from build123d import *

# Parameters (mm, degrees)
CUT_EXTRUDE1_START      = 8
CUT_EXTRUDE1_DEPTH      = 1.5
CUT_EXTRUDE2_DEPTH      = 140.867794721
CUT_EXTRUDE2_DEPTH_BACK = 140.867794721
SKETCH3_R               = 4


with BuildPart() as part:
    # Sketch1 → Revolve2 (revolve)
    with BuildSketch(Plane.XY, mode=Mode.PRIVATE) as revolve2_sk:
        Polygon((0, 8), (44, 8), (44, 10), (114, 10), (114, 11), (139, 11), (139, 4), (94, 4), (94, 0), (0, 0), align=None)
    revolve(revolve2_sk.sketch.rotate(Axis((0, 0, 0), (1, 0, 0)), 90), axis=Axis((0, 0, 0), (1, 0, 0)))

    # Sketch2 → Cut-Extrude1 (cut)
    with BuildSketch(Plane(origin=(0, 0, 0), x_dir=(1, 0, 0), z_dir=(0, 1, 0)).offset(CUT_EXTRUDE1_START)):
        with BuildLine():
            Line((23, 2), (41, 2))
            ThreePointArc((41, 2), (43, 0), (41, -2))
            Line((41, -2), (23, -2))
            ThreePointArc((23, -2), (21, 0), (23, 2))
        make_face()
    extrude(amount=-CUT_EXTRUDE1_DEPTH, mode=Mode.SUBTRACT)

    # Sketch3 → Cut-Extrude2 (cut, two sides: drawn at the far end of the back side and taken through both)
    with BuildSketch(Plane(origin=(0, 0, 0), x_dir=(1, 0, 0), z_dir=(0, 1, 0)).offset(-CUT_EXTRUDE2_DEPTH_BACK)):
        with Locations(Location((94, 0, 0), (0, 0, 270))):
            Circle(SKETCH3_R)
    extrude(amount=CUT_EXTRUDE2_DEPTH + CUT_EXTRUDE2_DEPTH_BACK, mode=Mode.SUBTRACT)


solid = part.part
The model under review builds one solid part; all positions refer to its coordinate system, in mm. A direction names the side the tool comes from. Give positions to 0.01 mm unless a question says otherwise; leave off trailing zeros. Order: outer loops, then holes, each group sorted by start corner. A loop starts at its lowest first (then second) coordinate and runs counter-clockwise, first axis right, second up. Notation, with made-up numbers: M 87.5,77.5 L 94.5,77.5 A16 cw 94.5,102.5 Z; hole C -17.75,19.5 d2. An arc over 180 degrees is marked long. Answer in a Markdown table with one row per item. Add a question column.
1. Add section B-B on y = 0. State the section outline as (x, z) points, plus the area to 3 significant figures.
2. For pin 1 Ø3 at (x, z) = (88, -4.5) entering from +Y; pin 2 Ø7 at (y, z) = (0, 0) entering from +X; pin 3 Ø9 at (x, z) = (94, 0) entering from -Y, all flat-tipped, find the tip position at first contact; note any pin that passes through.
3. Machinability: for faces 1 (the flat face through (0, 0, 0)), 2 (the flat face through (114, 10, -2)), 3 (the cylindrical face through (116.185, 1.532, 3.695)), which of the approach directions +Z, -Z, +X, -X, +Y, -Y give a long, thin tool a straight path to every point of the face, cutting with its end or side? Answer none if there is none.
4. Add section A-A on z = 0. State the section outline as (x, y) points, plus the area to 3 significant figures.
5. Mouldability with a two-part tool opening along X and no side actions: class faces 4 (the flat face through (44, -8.2, 0)), 5 (the flat face through (139, 5, 0)), 6 (the cylindrical face through (79.49, -3, 9.54)), 7 (the flat face through (32, 6.5, 0)) as released by +X, released by -X, zero draft, split by the parting line, or undercut.
6. To check wall thickness, follow line 1 along X through (y, z) = (-5.5, 0); line 2 along Z through (x, y) = (94, 0.5); line 3 along Y through (x, z) = (122.5, 0). State the ranges of each line that lie inside material, in increasing order.
7. Add section C-C on y = -6.25. State the section outline as (x, z) points.
8. Add section D-D on x = 83.5. State the section outline as (y, z) points.
The answers:
| question | item | result |
|---|---|---|
| 1 | outline | M 0,-8 L 44,-8 L 44,-10 L 114,-10 L 114,-11 L 139,-11 L 139,-4 L 94,-4 A4 cw 94,4 L 139,4 L 139,11 L 114,11 L 114,10 L 44,10 L 44,8 L 0,8 Z |
| 1 | area | 2,270 mm2 |
| 2 | pin 1 | y = 9.54 |
| 2 | pin 2 | x = 92.06 |
| 2 | pin 3 | y = -10 |
| 3 | face 1 | +Z, -Z, -X, +Y, -Y |
| 3 | face 2 | -X |
| 3 | face 3 | +X |
| 4 | outline | M 0,-8 L 44,-8 L 44,-10 L 90,-10 L 90,10 L 44,10 L 44,8 L 43,8 L 43,6.5 L 21,6.5 L 21,8 L 0,8 Z; M 98,-10 L 114,-10 L 114,-11 L 139,-11 L 139,-4 L 98,-4 Z; M 98,4 L 139,4 L 139,11 L 114,11 L 114,10 L 98,10 Z |
| 4 | area | 2,130 mm2 |
| 5 | face 4 | released by -X |
| 5 | face 5 | released by +X |
| 5 | face 6 | zero draft |
| 5 | face 7 | undercut |
| 6 | line 1 | 0 to 90, 98 to 139 |
| 6 | line 2 | -9.99 to -4, 4 to 9.99 |
| 6 | line 3 | -11 to -4, 4 to 11 |
| 7 | outline | M 0,-4.99 L 44,-4.99 L 44,-7.81 L 114,-7.81 L 114,-9.05 L 139,-9.05 L 139,9.05 L 114,9.05 L 114,7.81 L 44,7.81 L 44,4.99 L 0,4.99 Z; hole C 94,0 d8 |
| 8 | outline | C 0,0 d20 |
